Can you work these out from the model? Positions are in its coordinate system, mm. A direction names the side the tool comes from. Round coordinates to 2 decimals unless told otherwise and drop trailing zeros. Loops run counter-clockwise (first coordinate to the right, second up) from the corner with the lowest first, then second, coordinate; pieces in that order, holes last.
```python
from build123d import *

# Parameters (mm, degrees)
BOSS_EXTRUDE1_DEPTH  = 12
FILLET1_R            = 5
M5_CLEARANCE_HOLE1_D = 5.5
M5_CLEARANCE_HOLE2_D = 5.5


with BuildPart() as part:
    # Sketch1 → Boss-Extrude1 (new body)
    with BuildSketch(Plane(origin=(0, 0, 0), x_dir=(0, 0, -1), z_dir=(1, 0, 0))):
        Polygon((0, 0), (0, 50), (10, 50), (10, 10), (50, 10), (50, 0), align=None)
    extrude(amount=BOSS_EXTRUDE1_DEPTH)

    # Fillet1
    fillet1_edges = [part.edges().sort_by_distance(p)[0] for p in [
        (6, 10, -10),
    ]]
    fillet(fillet1_edges, radius=FILLET1_R)

    # M5 Clearance Hole1 (through all)
    with Locations(Plane(origin=(0, 0, -10), x_dir=(-1, 0, 0), z_dir=(0, 0, -1))):
        with Locations((-6, 25), (-6, 45)):
            Hole(M5_CLEARANCE_HOLE1_D / 2)

    # M5 Clearance Hole2 (through all)
    with Locations(Plane(origin=(0, 10, 0), x_dir=(1, 0, 0), z_dir=(0, 1, 0))):
        with Locations((6, 45), (6, 25)):
            Hole(M5_CLEARANCE_HOLE2_D / 2)


solid = part.part
```
(1) If I drill on line 1 (Z direction, x = 6, y = 3.25); line 2 (Y direction, x = 6, z = -3.5); line 3 (X direction, y = 6.25, z = -45), over which ranges is the centre line in solid material (lowest first)?
(2) Suppose I cut it at D-D (x = 10.5). Write out the boundary of the cut face in (y, z).
(3) For pin 1 (3.5 mm diameter, centred on x = 8, y = 25.5, fed in from -Z); pin 2 (5 mm diameter, centred on x = 6, y = 25, fed in from -Z); pin 3 (6 mm diameter, centred on x = 6, z = -29.5, fed in from +Y), each with a flat end and sliding along its axis, tell me the tip position at first contact or that it passes through.
(4) Which directions (+Z, -Z, +X, -X, +Y, -Y) give clear straight access to the entire face, cutting with the end or side of a thin tool? Please do faces 5 (the flat face through (0, 14, -9)), 6 (the flat face through (6, 33, -10)).
(5) Suppose I cut it at B-B (x = 6). Write out the boundary of the cut face in (y, z).
(6) Suppose I cut it at C-C (y = 45). Write out the boundary of the cut face in (x, z), then the cut area to 3 significant figures.
(7) Suppose I cut it at A-A (z = -45). Write out the boundary of the cut face in (x, y).
(8) We'd pull the mould along X, two halves only. Please class faces 1 (the cylindrical face through (5.642, 27.727, -4.93)), 2 (the flat face through (12, 14, -9)), 3 (the flat face through (6, 5, -50)), 4 (the cylindrical face through (6.358, 4.93, -27.727)): released by +X, released by -X, zero draft, split by the parting line, or undercut.
Check result:
1. line 1: z = -50 to -47.75, -42.25 to -27.75, -22.25 to 0
1. line 2: y = 0 to 22.25, 27.75 to 42.25, 47.75 to 50
1. line 3: x = 0 to 3.25, 8.75 to 12
2. outline: (0, -50) - (10, -50) - (10, -15) arc R5 cw to (15, -10) - (50, -10) - (50, 0) - (0, 0) - close
3. pin 1: stops at z = -10
3. pin 2: passes through
3. pin 3: stops at y = 10
4. face 5: +Z, -Z, -X, +Y, -Y
4. face 6: -Z, +X, -X, +Y
5. outline: (0, -50) - (10, -50) - (10, -47.75) - (0, -47.75) - close; (0, -42.25) - (10, -42.25) - (10, -27.75) - (0, -27.75) - close; (0, -22.25) - (10, -22.25) - (10, -15) arc R5 cw to (15, -10) - (22.25, -10) - (22.25, 0) - (0, 0) - close; (27.75, -10) - (42.25, -10) - (42.25, 0) - (27.75, 0) - close; (47.75, -10) - (50, -10) - (50, 0) - (47.75, 0) - close
6. outline: (0, -10) - (3.25, -10) - (3.25, 0) - (0, 0) - close; (8.75, -10) - (12, -10) - (12, 0) - (8.75, 0) - close
6. area: 65.0 mm2
7. outline: (0, 0) - (3.25, 0) - (3.25, 10) - (0, 10) - close; (8.75, 0) - (12, 0) - (12, 10) - (8.75, 10) - close
8. face 1: undercut
8. face 2: released by +X
8. face 3: zero draft
8. face 4: undercut
